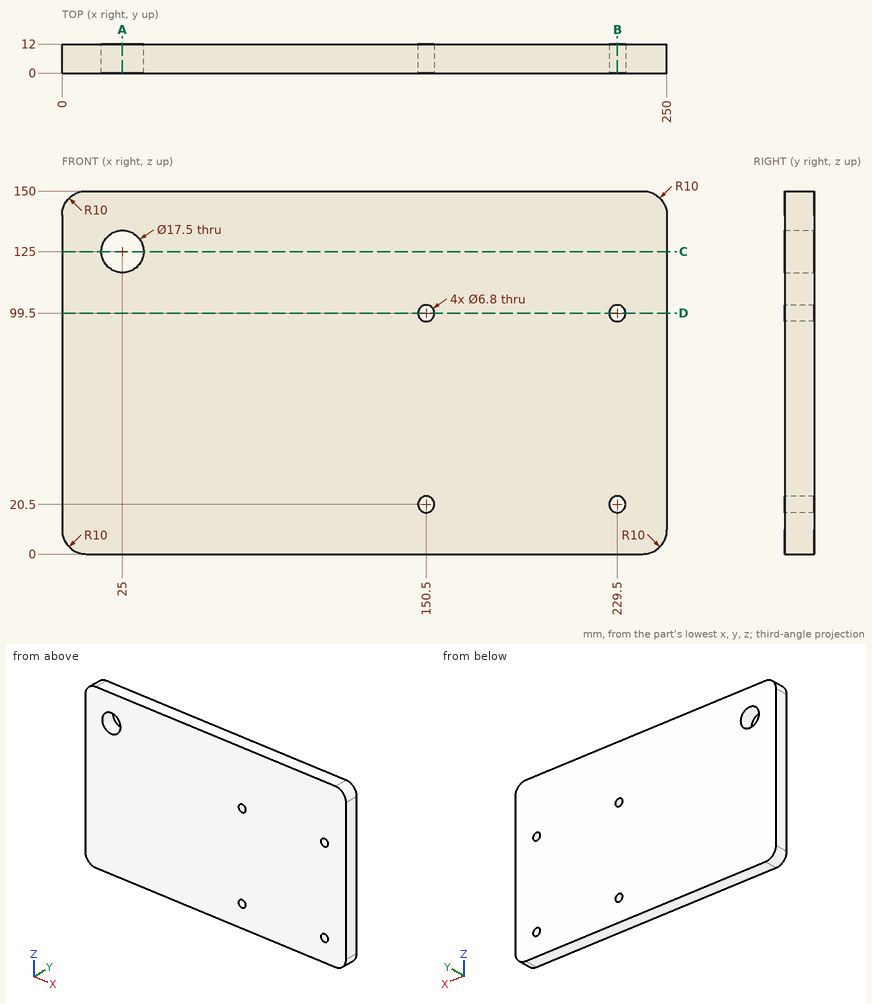
Answer from the drawing. Dimensions are ordinates in mm from the lowest x, y and z of the part. Round coordinates to 2 decimals unless told otherwise and drop trailing zeros. Loops run counter-clockwise (first coordinate to the right, second up) from the corner with the lowest first, then second, coordinate; pieces in that order, holes last.
(1) The part is cut by section D-D, the plane z = 99.5. Give the vertices of the cut face in (x, y), and give its area (3 significant figures).
Computed values:
outline: (0, 0) - (147.1, 0) - (147.1, 12) - (0, 12) - close; (153.9, 0) - (226.1, 0) - (226.1, 12) - (153.9, 12) - close; (232.9, 0) - (250, 0) - (250, 12) - (232.9, 12) - close
area: 2,840 mm2
(2) This flat-tipped pin is pushed along its axis until it touches: P1, Ø4, axis at x = 150.5, z = 99.5, coming from the +Y side. Where does it stop, or does it pass through?
Computed values:
P1: passes through
(3) The part is cut by section C-C, the plane z = 125. Give the vertices of the cut face in (x, y), and give its area (3 significant figures).
Computed values:
outline: (0, 0) - (16.25, 0) - (16.25, 12) - (0, 12) - close; (33.75, 0) - (250, 0) - (250, 12) - (33.75, 12) - close
area: 2,790 mm2
(4) The part is cut by section A-A, the plane x = 25. Give the vertices of the cut face in (y, z).
Computed values:
outline: (0, 0) - (12, 0) - (12, 116.25) - (0, 116.25) - close; (0, 133.75) - (12, 133.75) - (12, 150) - (0, 150) - close
(5) Find the intervals of material crossed by L1, parallel to Z at x = 229.5, y = 4.25; L2, parallel to X at y = 6.75, z = 99.5; L3, parallel to Z at x = 25, y = 6.5, in increasing order.
Computed values:
L1: z = 0 to 17.1, 23.9 to 96.1, 102.9 to 150
L2: x = 0 to 147.1, 153.9 to 226.1, 232.9 to 250
L3: z = 0 to 116.25, 133.75 to 150
(6) The part is cut by section B-B, the plane x = 229.5. Give the vertices of the cut face in (y, z), and give its area (3 significant figures).
Computed values:
outline: (0, 0) - (12, 0) - (12, 17.1) - (0, 17.1) - close; (0, 23.9) - (12, 23.9) - (12, 96.1) - (0, 96.1) - close; (0, 102.9) - (12, 102.9) - (12, 150) - (0, 150) - close
area: 1,640 mm2
